```python
from build123d import *

# Parameters (mm, degrees)
EXTRUDE_THIN1_DEPTH = 413.5


with BuildPart() as part:
    # Sketch1 → Extrude-Thin1 (new, symmetric)
    with BuildSketch(Plane(origin=(0, 0, 0), x_dir=(1, 0, 0), z_dir=(0, 1, 0))):
        with BuildLine():
            Line((-75, -25), (-75, 15))
            ThreePointArc((-75, 15), (-72.071067812, 22.071067812), (-65, 25))
            Line((-65, 25), (65, 25))
            ThreePointArc((65, 25), (72.071067812, 22.071067812), (75, 15))
            Line((75, 15), (75, -25))
            Line((75, -25), (72, -25))
            Line((72, -25), (72, 15))
            ThreePointArc((72, 15), (69.949747468, 19.949747468), (65, 22))
            Line((65, 22), (-65, 22))
            ThreePointArc((-65, 22), (-69.949747468, 19.949747468), (-72, 15))
            Line((-72, 15), (-72, -25))
            Line((-72, -25), (-75, -25))
        make_face()
    extrude(amount=EXTRUDE_THIN1_DEPTH, both=True)


solid = part.part
```
Model file for the job. Use its own axes, mm. A direction names the side the tool comes from. Give positions to 0.01 mm unless a question says otherwise; leave off trailing zeros. Write each loop counter-clockwise with the first axis right and the second up, starting at its lowest first coordinate (ties: lowest second). Pieces come first, ordered by that corner, then holes. Notation, with made-up numbers: M 65,50.25 L 77,50.25 A28 cw 77,68.25 Z; hole C -40,29.5 d11. An arc over 180 degrees is marked long. Use a Markdown table: item, result.
1) Cut at B-B (y = 30). List the corners of the cut face in (x, z).
Responses:
| item | result |
|---|---|
| outline | M -75,-15 A10 ccw -65,-25 L 65,-25 A10 ccw 75,-15 L 75,25 L 72,25 L 72,-15 A7 cw 65,-22 L -65,-22 A7 cw -72,-15 L -72,25 L -75,25 Z |
2) Cut at C-C (x = -35.5). List the corners of the cut face in (y, z), and give its area (3 significant figures).
Responses:
| item | result |
|---|---|
| outline | M -413.5,-25 L 413.5,-25 L 413.5,-22 L -413.5,-22 Z |
| area | 2,480 mm2 |
3) Drill centre lines: line 1 (X direction, y = -66, z = -4.5); line 2 (Z direction, x = -45, y = -265); line 3 (X direction, y = 219, z = -20). Where is each one in solid material? Low to high. Write a range as from..to.
Responses:
| item | result |
|---|---|
| line 1 | x = -75..-72, 72..75 |
| line 2 | z = -25..-22 |
| line 3 | x = -73.66..-69.9, 69.9..73.66 |
4) Pin check, flat tip, straight feed: pin 1 (2 mm diameter, centred on x = -28, y = -80, fed in from +Z). Stop position of the tip, or through.
Responses:
| item | result |
|---|---|
| pin 1 | stops at z = -22 |
5) Cut at A-A (z = 2.5). List the corners of the cut face in (x, y).
Responses:
| item | result |
|---|---|
| outline | M -75,-413.5 L -72,-413.5 L -72,413.5 L -75,413.5 Z; M 72,-413.5 L 75,-413.5 L 75,413.5 L 72,413.5 Z |
6) Tool access for faces 1 (the flat face through (75, 6, 5)), 2 (the flat face through (72, 6, 5)): list every direction of +Z, -Z, +X, -X, +Y, -Y with a clear straight run to the whole face (end or side of a thin tool).
Responses:
| item | result |
|---|---|
| face 1 | +Z, -Z, +X, +Y, -Y |
| face 2 | +Z, +Y, -Y |
